Geometry: final body of the model. Coordinates: model frame, mm. Face numbers are marked on the shaded views. Round coordinates to 2 decimals unless told otherwise and drop trailing zeros. Write each loop counter-clockwise with the first axis right and the second up, starting at its lowest first coordinate (ties: lowest second). Pieces come first, ordered by that corner, then holes. Notation, with made-up numbers: M 17.5,5 L 55.5,5 A26 cw 55.5,25 Z; hole C 67.5,38 d3. An arc over 180 degrees is marked long. Use one line per item in the form item = value. Start each with the question number.
Item 1: Pull-direction query (Y, two-part tool) for the marked faces 1, 2 and 3; classes: pulls with the +Y half, pulls with the -Y half, needs draft (parallel to the pull), parting line crosses it, or undercut.
Item 2: Section query C-C (z = -5.5). Return loops of the section in (x, y), and give its area (3 significant figures).
Item 3: Pin query (flat end, axial travel): pin 1 Ø5 at (x, z) = (583.5, -5.5) entering from -Y; pin 2 Ø3 at (y, z) = (-315, -3.5) entering from -X; pin 3 Ø1 at (y, z) = (-241.5, -5.5) entering from +X. Return the tip coordinate at first contact, or that it passes through.
Item 4: Section query D-D (x = 530). Return loops of the section in (y, z).
Item 5: Section query A-A (x = 565.5). Return loops of the section in (y, z), and give its area (3 significant figures).
Item 6: Ray query, probe 1 along X at (y, z) = (-297, -3.5); probe 2 along X at (y, z) = (-286, -7.25); probe 3 along Y at (x, z) = (553, -4). Return the intervals inside material, ascending.
Item 7: Section query B-B (y = -285). Return loops of the section in (x, z), and give its area (3 significant figures).
from build123d import *

# Parameters (mm, degrees)
SKETCH_2_R      = 17.5
EXTRUDE_1_DEPTH = 10


with BuildPart() as part:
    # 草图2 → 凸台-拉伸1 (new body)
    with BuildSketch(Plane.XY):
        with BuildLine():
            Line((507.065379812, -222.122666991), (535.409266278, -318.021697747))
            ThreePointArc((535.409266278, -318.021697747), (572.682141445, -338.288241034), (592.948684732, -301.015365867))
            Line((592.948684732, -301.015365867), (569.631184207, -222.122666991))
            Line((569.631184207, -222.122666991), (507.065379812, -222.122666991))
        make_face()
        with Locations((558.927759659, -291.75150785)):
            Circle(SKETCH_2_R, mode=Mode.SUBTRACT)
    extrude(amount=-EXTRUDE_1_DEPTH)


solid = part.part
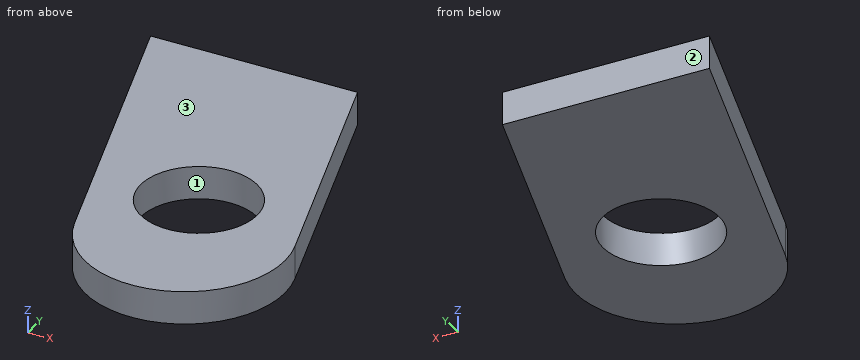
Working result:
q1.face_1 = undercut
q1.face_2 = pulls with the +Y half
q1.face_3 = needs draft
q2.outline = M 507.07,-222.12 L 535.41,-318.02 A30 ccw 592.95,-301.02 L 569.63,-222.12 Z; hole C 558.93,-291.75 d35
q2.area = 5,920 mm²
q3.pin_1 = -334.36
q3.pin_2 = 534.07
q3.pin_3 = 575.51
q4.outline = M -299.72,-10 L -222.12,-10 L -222.12,0 L -299.72,0 Z
q5.outline = M -339.49,-10 L -307.97,-10 L -307.97,0 L -339.49,0 Z; M -275.53,-10 L -222.12,-10 L -222.12,0 L -275.53,0 Z
q5.area = 849 mm²
q6.probe_1 = 529.2 to 542.23, 575.62 to 591.76
q6.probe_2 = 525.94 to 542.4, 575.46 to 588.51
q6.probe_3 = -337.36 to -308.22, -275.29 to -222.12
q7.outline = M 525.65,-10 L 542.78,-10 L 542.78,0 L 525.65,0 Z; M 575.07,-10 L 588.22,-10 L 588.22,0 L 575.07,0 Z
q7.area = 303 mm²
